```python
from build123d import *

# Parameters (mm, degrees)
BASE_PROFILE_SKETCH_W     = 29
BASE_PROFILE_SKETCH_H     = 32
BASE_BLOCK_DEPTH          = 16
CENTRE_SLOT_SKETCH_W      = 13
CENTRE_SLOT_SKETCH_H      = 10
CENTRE_SLOT_DEPTH         = 16
SIDE_NOTCH_SKETCH_W       = 9
SIDE_NOTCH_SKETCH_H       = 15
SIDE_NOTCH_DEPTH          = 27.874709301
FOOT_HOLE_SKETCH_R        = 3.5
FOOT_HOLE_DEPTH           = 37.783148315
UPRIGHT_LUG_1_DEPTH       = 7
UPRIGHT_LUG_2_SKETCH_W    = 8
UPRIGHT_LUG_2_SKETCH_H    = 16
UPRIGHT_LUG_2_DEPTH       = 7
LUG_1_CROSS_HOLE_SKETCH_R = 3.5
LUG_1_CROSS_HOLE_DEPTH    = 7
LUG_2_CROSS_HOLE_SKETCH_R = 3.5
LUG_2_CROSS_HOLE_DEPTH    = 7


with BuildPart() as part:
    # Base Profile Sketch → Base Block (new body)
    with BuildSketch(Plane.XY):
        Rectangle(BASE_PROFILE_SKETCH_W, BASE_PROFILE_SKETCH_H)
    extrude(amount=BASE_BLOCK_DEPTH)

    # Centre Slot Sketch → Centre Slot (cut)
    with BuildSketch(Plane.XY.offset(16)):
        with Locations((0, -11)):
            Rectangle(CENTRE_SLOT_SKETCH_W, CENTRE_SLOT_SKETCH_H)
    extrude(amount=-CENTRE_SLOT_DEPTH, mode=Mode.SUBTRACT)

    # Side Notch Sketch → Side Notch (cut, through all)
    with BuildSketch(Plane.XY.offset(16)):
        with Locations((0, 8.5)):
            Rectangle(SIDE_NOTCH_SKETCH_W, SIDE_NOTCH_SKETCH_H)
    extrude(amount=-SIDE_NOTCH_DEPTH, mode=Mode.SUBTRACT)

    # Foot Hole Sketch → Foot Hole (cut, through all)
    with BuildSketch(Plane(origin=(14.5, 0, 0), x_dir=(0, 0, -1), z_dir=(1, 0, 0))):
        with Locations((-8, 9)):
            Circle(FOOT_HOLE_SKETCH_R)
    extrude(amount=-FOOT_HOLE_DEPTH, mode=Mode.SUBTRACT)

    # Upright Lug 1 Sketch → Upright Lug 1 (add)
    with BuildSketch(Plane.XZ.offset(16)):
        Polygon((-18.5, 0), (-24.5, 6), (-24.5, 16), (-14.5, 16), (-6.5, 16), (-6.5, 0), (-14.5, 0), align=None)
    extrude(amount=-UPRIGHT_LUG_1_DEPTH)

    # Upright Lug 2 Sketch → Upright Lug 2 (add)
    with BuildSketch(Plane.XZ.offset(16)):
        Polygon((14.5, 0), (18.5, 0), (24.5, 6), (24.5, 16), (14.5, 16), align=None)
        with Locations((10.5, 8)):
            Rectangle(UPRIGHT_LUG_2_SKETCH_W, UPRIGHT_LUG_2_SKETCH_H)
    extrude(amount=-UPRIGHT_LUG_2_DEPTH)

    # Lug 1 Cross Hole Sketch → Lug 1 Cross Hole (cut)
    with BuildSketch(Plane(origin=(0, -9, 0), x_dir=(1, 0, 0), z_dir=(0, 1, 0))):
        with Locations(Location((-19.5, -8, 0), (0, 0, 270))):
            Circle(LUG_1_CROSS_HOLE_SKETCH_R)
    extrude(amount=-LUG_1_CROSS_HOLE_DEPTH, mode=Mode.SUBTRACT)

    # Lug 2 Cross Hole Sketch → Lug 2 Cross Hole (cut)
    with BuildSketch(Plane(origin=(0, -9, 0), x_dir=(1, 0, 0), z_dir=(0, 1, 0))):
        with Locations(Location((19.5, -8, 0), (0, 0, 270))):
            Circle(LUG_2_CROSS_HOLE_SKETCH_R)
    extrude(amount=-LUG_2_CROSS_HOLE_DEPTH, mode=Mode.SUBTRACT)


solid = part.part
```
Model file for the job. Use its own axes, mm. A direction names the side the tool comes from. Round coordinates to 2 decimals unless told otherwise and drop trailing zeros. Write each loop counter-clockwise with the first axis right and the second up, starting at its lowest first coordinate (ties: lowest second). Pieces come first, ordered by that corner, then holes. Notation, with made-up numbers: M 35.25,39.25 L 90.25,39.25 A10 cw 90.25,45.25 Z; hole C 40,-31 d7. An arc over 180 degrees is marked long. Put each result on its own line as item: value.
Item 1: Cut at D-D (z = 10.75). State how many separate pieces and enclosed holes the cut face has, and give its area (3 significant figures).
Responses:
separate pieces: 5
enclosed holes: 0
area: 656 mm²
Item 2: Cut at B-B (x = 19.5). List the corners of the cut face in (y, z).
Responses:
outline: M -16,1 L -9,1 L -9,4.5 L -16,4.5 Z; M -16,11.5 L -9,11.5 L -9,16 L -16,16 Z
Item 3: Probe L1, parallel to X at y = -12.5, z = 8; L2, parallel to X at y = 10.5, z = 1; L3, parallel to X at y = -13.5, z = 9.5. List the from-to ranges inside material, lowest first. Write a range as from..to.
Responses:
L1: -24.5..-23, -16..-6.5, 6.5..16, 23..24.5
L2: -14.5..-4.5, 4.5..14.5
L3: -24.5..-22.66, -16.34..-6.5, 6.5..16.34, 22.66..24.5
Item 4: Cut at C-C (y = 9). List the corners of the cut face in (x, z).
Responses:
outline: M -14.5,0 L -4.5,0 L -4.5,4.5 L -14.5,4.5 Z; M -14.5,11.5 L -4.5,11.5 L -4.5,16 L -14.5,16 Z; M 4.5,0 L 14.5,0 L 14.5,4.5 L 4.5,4.5 Z; M 4.5,11.5 L 14.5,11.5 L 14.5,16 L 4.5,16 Z
Item 5: Mould opens along Z. For faces 4 (the flat face through (-4.5, 5, 8)), 5 (the flat face through (0, 0, 16)), 6 (the flat face through (-21.5, -12.5, 3)), 7 (the cylindrical face through (21.865, -12.451, 5.42)) say: +Z half, -Z half, draft (parallel to the pull), parting line (faces both ways), or undercut.
Responses:
face 4: draft
face 5: +Z half
face 6: -Z half
face 7: undercut
Item 6: Flat gauge pins, fed straight in: P1, Ø4.5, axis at x = -1.5, z = 9.5, coming from the +Y side; P2, Ø8, axis at x = -20.5, z = 4.5, coming from the +Y side; P3, Ø4, axis at x = 0.5, z = 10, coming from the -Y side. Where does each tip first touch, or does it go through?
Responses:
P1: y = 1
P2: y = -9
P3: y = -6
Item 7: Tool access for faces 1 (the flat face through (0, 1, 8)), 2 (the flat face through (6.5, -11, 8)), 3 (the flat face through (-14.5, 3, 8)): list every direction of +Z, -Z, +X, -X, +Y, -Y with a clear straight run to the whole face (end or side of a thin tool).
Responses:
face 1: +Z, -Z, +Y
face 2: +Z, -Z, -Y
face 3: +Z, -Z, -X, +Y
Item 8: Cut at A-A (y = -11). List the corners of the cut face in (x, z), and give its area (3 significant figures).
Responses:
outline: M -24.5,6 L -18.5,0 L -6.5,0 L -6.5,16 L -24.5,16 Z; M 6.5,0 L 18.5,0 L 24.5,6 L 24.5,16 L 6.5,16 Z; hole C -19.5,8 d7; hole C 19.5,8 d7
area: 463 mm²
